```python
from build123d import *

# Parameters (mm, degrees)
SKETCH1_W              = 22
SKETCH1_H              = 22
BOSS_EXTRUDE1_DEPTH    = 16
M10_TAPPED_HOLE1_D     = 8.5
M10_TAPPED_HOLE1_DEPTH = 27.5
M10_TAPPED_HOLE1_TIP   = 2.553657631


with BuildPart() as part:
    # Sketch1 → Boss-Extrude1 (new body)
    with BuildSketch(Plane.XY):
        Rectangle(SKETCH1_W, SKETCH1_H)
    extrude(amount=BOSS_EXTRUDE1_DEPTH)

    # M10 Tapped Hole1
    with Locations(Plane.XY.offset(16)):
        with Locations((0, 0)):
            Hole(M10_TAPPED_HOLE1_D / 2, depth=M10_TAPPED_HOLE1_DEPTH)
            with Locations((0, 0, -(M10_TAPPED_HOLE1_DEPTH + M10_TAPPED_HOLE1_TIP / 2))):  # 118° drill point
                Cone(0, M10_TAPPED_HOLE1_D / 2, M10_TAPPED_HOLE1_TIP, mode=Mode.SUBTRACT)


solid = part.part
```
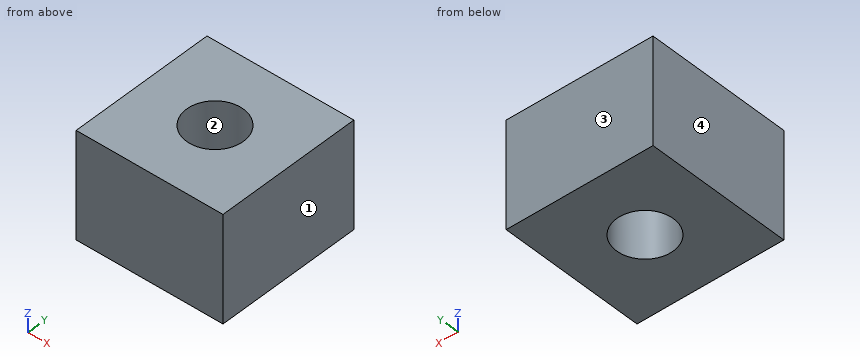
Work out the finished part from the listing and answer in its coordinate system (mm). Face numbers are marked on the shaded views. Coordinates: 2 decimals unless noted, no trailing zeros. Order: outer loops, then holes, each group sorted by start corner. A loop starts at its lowest first (then second) coordinate and runs counter-clockwise, first axis right, second up. Notation, with made-up numbers: M 81.25,57.5 L 87.25,57.5 A16 ccw 87.25,61.5 Z; hole C -3,70.5 d7. An arc over 180 degrees is marked long. Use CSV: the item, a comma, the result in double quotes.
1) Section C-C on z = 7 is taken. Write down the section's boundary in (x, y).
Worked out:
outline,"M -11,-11 L 11,-11 L 11,11 L -11,11 Z; hole C 0,0 d8.5"
2) Section A-A on y = 0 is taken. Write down the section's boundary in (x, z).
Worked out:
outline,"M -11,0 L -4.25,0 L -4.25,16 L -11,16 Z; M 4.25,0 L 11,0 L 11,16 L 4.25,16 Z"
3) Determine the mould class of the marked faces 1, 2, 3 and 4 for opening direction X: released by +X, released by -X, zero draft, split by the parting line, or undercut.
Worked out:
face 1,"released by +X"
face 2,"undercut"
face 3,"zero draft"
face 4,"released by -X"
4) Consider line 1 (Y direction, x = 0, z = 11.25); line 2 (Y direction, x = 3, z = 11.25); line 3 (X direction, y = 3.5, z = 6.5). Determine where each line is inside the solid, lowest interval first. Write a range as [from, to].
Worked out:
line 1,"y = [-11, -4.25], [4.25, 11]"
line 2,"y = [-11, -3.01], [3.01, 11]"
line 3,"x = [-11, -2.41], [2.41, 11]"
